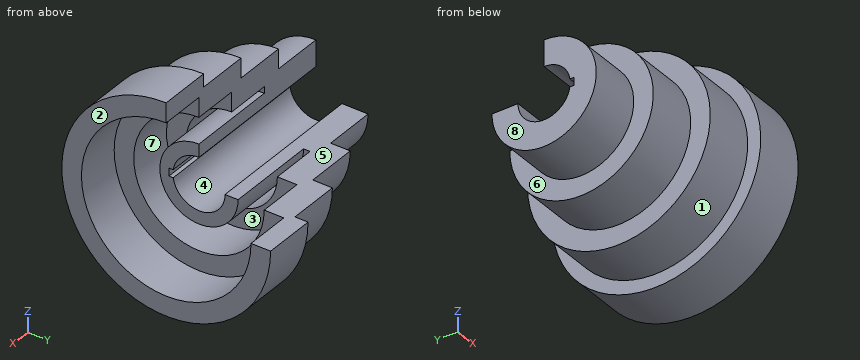
from build123d import *

# Parameters (mm, degrees)
STEPPED_PULLEY_BODY_ANGLE  = 270
KEYWAY_SLOT_6X3_DEPTH      = 196.959179423
KEYWAY_SLOT_6X3_DEPTH_BACK = 196.959179423


with BuildPart() as part:
    # Pulley Profile Sketch → Stepped Pulley Body (revolve)
    with BuildSketch(Plane.XY):
        Polygon((0, 40), (0, 20), (125, 20), (125, 30), (55, 30), (55, 35), (90, 35), (90, 50), (125, 50), (125, 65), (160, 65), (160, 80), (120, 80), (120, 70), (80, 70), (80, 55), (40, 55), (40, 40), align=None)
    revolve(axis=Axis((125, 0, 0), (-1, 0, 0)), revolution_arc=STEPPED_PULLEY_BODY_ANGLE)

    # Keyway Slot Sketch → Keyway Slot 6x3 (cut, two sides: drawn at the far end of the back side and taken through both)
    with BuildSketch(Plane(origin=(0, 0, 0), x_dir=(0, 0, -1), z_dir=(1, 0, 0)).offset(-KEYWAY_SLOT_6X3_DEPTH_BACK)):
        with BuildLine():
            ThreePointArc((3, -19.773719933), (1.504260837, -19.943349752), (0, -20))
            Line((0, -20), (0, -23))
            Line((0, -23), (3, -23))
            Line((3, -23), (3, -19.773719933))
        make_face()
        with BuildLine():
            Line((0, -23), (0, -20))
            ThreePointArc((0, -20), (-1.504260837, -19.943349752), (-3, -19.773719933))
            Line((-3, -19.773719933), (-3, -23))
            Line((-3, -23), (0, -23))
        make_face()
    extrude(amount=KEYWAY_SLOT_6X3_DEPTH + KEYWAY_SLOT_6X3_DEPTH_BACK, mode=Mode.SUBTRACT)


solid = part.part
Could you check a few things on this model? Use its own coordinates, in mm. Face numbers are marked on the shaded views. A direction names the side the tool comes from. Give positions to 0.01 mm unless a question says otherwise; leave off trailing zeros. Write each loop counter-clockwise with the first axis right and the second up, starting at its lowest first coordinate (ties: lowest second). Pieces come first, ordered by that corner, then holes. Notation, with made-up numbers: (21, 4.5) -> (36, 4.5) arc R16 cw to (36, 34.5) -> close; hole circle Ø9 at (31, 4). An arc over 180 degrees is marked (long way). Answer as a JSON object with one key per item and string values.
Q1. Which directions (+Z, -Z, +X, -X, +Y, -Y) give clear straight access to the entire face, cutting with the end or side of a thin tool? Please do the marked faces 4, 5, 6, 7 and 8.
Taken from the geometry:
{"face 4": "+X, -X", "face 5": "+Z, +X, -X, +Y", "face 6": "-X", "face 7": "+X", "face 8": "+Z, -Z, -X, +Y, -Y"}
Q2. Will these pins go through, and if not, where does the flat tip stop? pin 1 Ø1.8 at (x, z) = (88, 0) entering from +Y; pin 2 Ø18 at (y, z) = (7, 8) entering from +X; pin 3 Ø1 at (x, y) = (59, 2) entering from +Z; pin 4 Ø5 at (x, z) = (27.5, 21) entering from -Y.
Taken from the geometry:
{"pin 1": "stops at y = 70", "pin 2": "passes through", "pin 3": "stops at z = -19.84", "pin 4": "stops at y = -35.46"}
Q3. We'd pull the mould along Y, two halves only. Please class the marked faces 1, 2 and 3: released by +Y, released by -Y, zero draft, split by the parting line, or undercut.
Taken from the geometry:
{"face 1": "split by the parting line", "face 2": "zero draft", "face 3": "undercut"}
Q4. Suppose I cut it at C-C on y = 45.5. Write out the boundary of the cut face in (x, z).
Taken from the geometry:
{"outline": "(40, -30.9) -> (80, -30.9) -> (80, -53.2) -> (120, -53.2) -> (120, -65.8) -> (160, -65.8) -> (160, -46.42) -> (125, -46.42) -> (125, -20.73) -> (90, -20.73) -> (90, 0) -> (40, 0) -> close"}
Q5. Please list where these lines run through material, in increasing order: L1, parallel to Z at x = 68.5, y = -4.5; L2, parallel to X at y = -57, z = -29; L3, parallel to Z at x = 118.5, y = -5.
Taken from the geometry:
{"L1": "z = -54.82 to -34.71, -29.66 to -19.49, 19.49 to 29.66, 34.71 to 54.82", "L2": "x = 80 to 125", "L3": "z = -69.82 to -49.75, -29.58 to -19.36, 19.36 to 29.58, 49.75 to 69.82"}
Q6. Suppose I cut it at D-D on z = 9. Write out the boundary of the cut face in (x, y).
Taken from the geometry:
{"outline": "(0, -38.97) -> (40, -38.97) -> (40, -54.26) -> (80, -54.26) -> (80, -69.42) -> (120, -69.42) -> (120, -79.49) -> (160, -79.49) -> (160, -64.37) -> (125, -64.37) -> (125, -49.18) -> (90, -49.18) -> (90, -33.82) -> (55, -33.82) -> (55, -28.62) -> (125, -28.62) -> (125, -17.86) -> (0, -17.86) -> close"}
Q7. Suppose I cut it at B-B on x = 34.5. Write out the boundary of the cut face in (y, z), then the cut area to 3 significant figures.
Taken from the geometry:
{"outline": "(-23, -3) -> (-23, 3) -> (-19.77, 3) arc R20 cw to (0, 20) -> (0, 40) arc R40 ccw (long way) to (40, 0) -> (20, 0) arc R20 cw to (-19.77, -3) -> close", "area": "2,810 mm²"}
Q8. Suppose I cut it at A-A on x = 86.5. Write out the boundary of the cut face in (y, z), then the cut area to 3 significant figures.
Taken from the geometry:
{"outline": "(-23, -3) -> (-23, 3) -> (-19.77, 3) arc R20 cw to (0, 20) -> (0, 30) arc R30 ccw (long way) to (30, 0) -> (20, 0) arc R20 cw to (-19.77, -3) -> close; (0, 35) -> (0, 70) arc R70 ccw (long way) to (70, 0) -> (35, 0) arc R35 cw (long way) to start", "area": "9,820 mm²"}
